```python
from build123d import *

# Parameters (mm, degrees)
SKETCH_1_W          = 95
SKETCH_1_H          = 18
EXTRUDE_1_DEPTH     = 6
SKETCH_2_R          = 5
CUT_EXTRUDE_1_DEPTH = 6
SKETCH_5_R          = 3
CUT_EXTRUDE_3_DEPTH = 10
SKETCH_6_W          = 6
SKETCH_6_H          = 18
EXTRUDE_3_DEPTH     = 25
SKETCH_7_W          = 6
SKETCH_7_H          = 18
EXTRUDE_4_DEPTH     = 30
SKETCH_8_R          = 2
CUT_EXTRUDE_4_DEPTH = 20


with BuildPart() as part:
    # 草图1 → 凸台-拉伸1 (new body)
    with BuildSketch(Plane.XY):
        Rectangle(SKETCH_1_W, SKETCH_1_H)
    extrude(amount=EXTRUDE_1_DEPTH)

    # 草图2 → 切除-拉伸1 (cut)
    with BuildSketch(Plane.XY.offset(6)):
        with Locations((-35.5, 0)):
            Circle(SKETCH_2_R)
        with Locations((14.5, 0)):
            Circle(SKETCH_2_R)
    extrude(amount=-CUT_EXTRUDE_1_DEPTH, mode=Mode.SUBTRACT)

    # 草图5 → 切除-拉伸3 (cut)
    with BuildSketch(Plane(origin=(0, 0, 0), x_dir=(-1, 0, 0), z_dir=(0, 0, -1))):
        with Locations((-32.5, 0)):
            Circle(SKETCH_5_R)
    extrude(amount=-CUT_EXTRUDE_3_DEPTH, mode=Mode.SUBTRACT)

    # 草图6 → 凸台-拉伸3 (add)
    with BuildSketch(Plane(origin=(47.5, 0, 0), x_dir=(0, 0, -1), z_dir=(1, 0, 0))):
        with Locations((-3, 0)):
            Rectangle(SKETCH_6_W, SKETCH_6_H)
    extrude(amount=EXTRUDE_3_DEPTH)

    # 草图7 → 凸台-拉伸4 (add)
    with BuildSketch(Plane.XY.offset(6)):
        with Locations((69.5, 0)):
            Rectangle(SKETCH_7_W, SKETCH_7_H)
    extrude(amount=EXTRUDE_4_DEPTH)

    # 草图8 → 切除-拉伸4 (cut)
    with BuildSketch(Plane(origin=(72.5, 0, 0), x_dir=(0, 0, -1), z_dir=(1, 0, 0))):
        with Locations((-25, 0)):
            Circle(SKETCH_8_R)
    extrude(amount=-CUT_EXTRUDE_4_DEPTH, mode=Mode.SUBTRACT)


solid = part.part
```
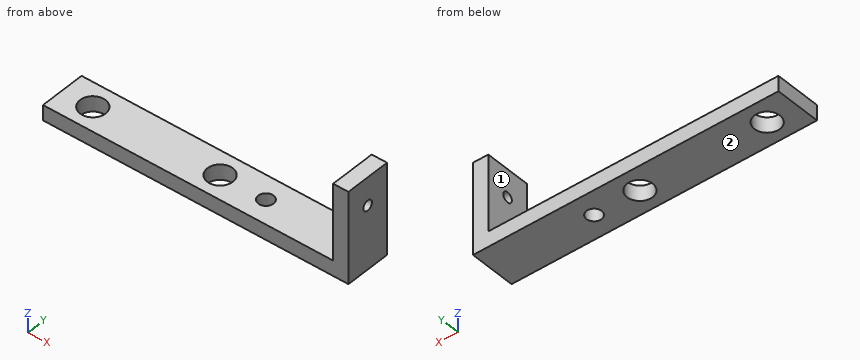
Here's how the part is built. I have some questions about the finished solid (model axes, mm). Face numbers are marked on the shaded views. A direction names the side the tool comes from. Coordinates: 2 decimals unless noted, no trailing zeros. Order: outer loops, then holes, each group sorted by start corner. A loop starts at its lowest first (then second) coordinate and runs counter-clockwise, first axis right, second up.
1) Imagine slicing it at D-D on y = -7.5. List the corners of the cut face in (x, z) for me, and give its area (3 significant figures).
2) Imagine slicing it at C-C on z = 25. List the corners of the cut face in (x, y) for me, and give its area (3 significant figures).
3) Imagine slicing it at B-B on y = 0. List the corners of the cut face in (x, z) for me, and give its area (3 significant figures).
4) I need wall thicknesses on line 1 (Y direction, x = 69.95, z = 25); line 2 (Y direction, x = 14.5, z = 4.35); line 3 (Z direction, x = -9.5, y = -2.5). Which ranges of each line are inside material? Lowest first, please.
5) Will these pins go through, and if not, where does the flat tip stop? pin 1 (1 mm diameter, centred on x = -29, y = 2.5, fed in from +Z); pin 2 (5.5 mm diameter, centred on y = -2, z = 19, fed in from -X).
6) Which directions (+Z, -Z, +X, -X, +Y, -Y) give clear straight access to the entire face, cutting with the end or side of a thin tool? Please do the marked faces 1 and 2.
7) Imagine slicing it at A-A on x = 14.5. List the corners of the cut face in (y, z) for me, and give its area (3 significant figures).
Response values:
1. outline: (-47.5, 0) - (72.5, 0) - (72.5, 36) - (66.5, 36) - (66.5, 6) - (-47.5, 6) - close
1. area: 900 mm2
2. outline: (66.5, -9) - (72.5, -9) - (72.5, -2) - (66.5, -2) - close; (66.5, 2) - (72.5, 2) - (72.5, 9) - (66.5, 9) - close
2. area: 84.0 mm2
3. outline: (-47.5, 0) - (-40.5, 0) - (-40.5, 6) - (-47.5, 6) - close; (-30.5, 0) - (9.5, 0) - (9.5, 6) - (-30.5, 6) - close; (19.5, 0) - (29.5, 0) - (29.5, 6) - (19.5, 6) - close; (35.5, 0) - (72.5, 0) - (72.5, 23) - (66.5, 23) - (66.5, 6) - (35.5, 6) - close; (66.5, 27) - (72.5, 27) - (72.5, 36) - (66.5, 36) - close
3. area: 720 mm2
4. line 1: y = -9 to -2, 2 to 9
4. line 2: y = -9 to -5, 5 to 9
4. line 3: z = 0 to 6
5. pin 1: stops at z = 6
5. pin 2: stops at x = 66.5
6. face 1: +Z, -X, +Y, -Y
6. face 2: -Z, +X, -X, +Y, -Y
7. outline: (-9, 0) - (-5, 0) - (-5, 6) - (-9, 6) - close; (5, 0) - (9, 0) - (9, 6) - (5, 6) - close
7. area: 48.0 mm2
